Part model, mm, in its own coordinate system. A direction names the side the tool comes from. Coordinates: 2 decimals unless noted, no trailing zeros. Write each loop counter-clockwise with the first axis right and the second up, starting at its lowest first coordinate (ties: lowest second). Pieces come first, ordered by that corner, then holes. Notation, with made-up numbers: (68.5, 33.25) - (101.5, 33.25) arc R4 cw to (101.5, 37.25) - close; hole circle Ø9 at (88.5, -29). An arc over 180 degrees is marked (long way). Use a Markdown table: item, result.
```python
from build123d import *

# Parameters (mm, degrees)
BOSS_EXTRUDE1_DEPTH = 45
SKETCH2_R           = 1.5
CUT_EXTRUDE1_DEPTH  = 47.786750261
FILLET1_R           = 3


with BuildPart() as part:
    # Sketch1 → Boss-Extrude1 (new body)
    with BuildSketch(Plane.XY):
        with BuildLine():
            Line((0, 4), (0, 2))
            Line((0, 2), (-8, 2))
            Line((-8, 2), (-8, -2))
            Line((-8, -2), (0, -2))
            Line((0, -2), (0, -4))
            Line((0, -4), (-8, -4))
            ThreePointArc((-8, -4), (-9.414213562, -3.414213562), (-10, -2))
            Line((-10, -2), (-10, 2))
            ThreePointArc((-10, 2), (-9.414213562, 3.414213562), (-8, 4))
            Line((-8, 4), (0, 4))
        make_face()
    extrude(amount=BOSS_EXTRUDE1_DEPTH)

    # Sketch2 → Cut-Extrude1 (cut, through all)
    with BuildSketch(Plane(origin=(0, -4, 0), x_dir=(-1, 0, 0), z_dir=(0, -1, 0))):
        with Locations(Location((3, -3, 0), (0, 0, 180))):
            Circle(SKETCH2_R)
        with Locations(Location((3, -42, 0), (0, 0, 180))):
            Circle(SKETCH2_R)
    extrude(amount=-CUT_EXTRUDE1_DEPTH, mode=Mode.SUBTRACT)

    # Fillet1
    fillet1_edges = [part.edges().sort_by_distance(p)[0] for p in [
        (0, 3, 0),
        (0, -3, 0),
        (0, 3, 45),
        (0, -3, 45),
    ]]
    fillet(fillet1_edges, radius=FILLET1_R)


solid = part.part
```
Item 1: Which spindle directions (+Z, -Z, +X, -X, +Y, -Y) get a long thin tool onto all of the face, cutting with end or side? Do faces 5 (the face through (-9.43, 3.4, 22.18)), 6 (the face through (-4, 2, 22)). Say none if no direction does.
From the geometry:
| item | result |
|---|---|
| face 5 | +Z, -Z, -X, +Y |
| face 6 | +Z, -Z, +X |
Item 2: Two-plate mould, pull along X, no slides. Class faces 1 (the face through (-0.86, 2.99, 0.9)), 2 (the face through (-9, 0, 45)), 3 (the face through (-3.325, -3.014, 40.536)), 4 (the face through (-9.4, -3.43, 22.18)): pulls with the +X half, pulls with the -X half, needs draft (parallel to the pull), parting line crosses it, or undercut.
From the geometry:
| item | result |
|---|---|
| face 1 | pulls with the +X half |
| face 2 | needs draft |
| face 3 | undercut |
| face 4 | pulls with the -X half |
Item 3: Band-saw the part on D-D, the plane y = -0.75. Give the cut face in (x, z).
From the geometry:
| item | result |
|---|---|
| outline | (-10, 0) - (-8, 0) - (-8, 45) - (-10, 45) - close |
Item 4: Drop flat-ended pins along their axis: P1, Ø1.8, axis at x = -3, z = 42, coming from the +Y side (3 decimals); P2, Ø1, axis at x = -1, y = 2, coming from the +Z side. Give the stop position or say it passes through.
From the geometry:
| item | result |
|---|---|
| P1 | through |
| P2 | z = 44.6 |
Item 5: Band-saw the part on C-C, the plane y = -2.75. Give the cut face in (x, z).
From the geometry:
| item | result |
|---|---|
| outline | (-9.85, 0) - (-3, 0) arc R3 ccw to (0, 3) - (0, 42) arc R3 ccw to (-3, 45) - (-9.85, 45) - close; hole circle Ø3 at (-3, 3); hole circle Ø3 at (-3, 42) |
Item 6: Band-saw the part on B-B, the plane z = 27. Give the cut face in (x, y).
From the geometry:
| item | result |
|---|---|
| outline | (-10, -2) arc R2 ccw to (-8, -4) - (0, -4) - (0, -2) - (-8, -2) - (-8, 2) - (0, 2) - (0, 4) - (-8, 4) arc R2 ccw to (-10, 2) - close |
Item 7: Band-saw the part on A-A, the plane x = -5. Give the cut face in (y, z).
From the geometry:
| item | result |
|---|---|
| outline | (-4, 0) - (-2, 0) - (-2, 45) - (-4, 45) - close; (2, 0) - (4, 0) - (4, 45) - (2, 45) - close |
Item 8: Drill centre lines: probe 1 along Y at (x, z) = (-1, 21); probe 2 along Z at (x, y) = (-2, -3); probe 3 along Z at (x, y) = (-2.5, 3.5). Where is each one in solid material? Low to high.
From the geometry:
| item | result |
|---|---|
| probe 1 | -4 to -2, 2 to 4 |
| probe 2 | 0.17 to 1.88, 4.12 to 40.88, 43.12 to 44.83 |
| probe 3 | 0.04 to 1.59, 4.41 to 40.59, 43.41 to 44.96 |
